```python
from build123d import *

# Parameters (mm, degrees)
BOSS_EXTRUDE1_DEPTH = 10
M10_TAPPED_HOLE1_D  = 8.5


with BuildPart() as part:
    # Sketch1 → Boss-Extrude1 (new body)
    with BuildSketch(Plane(origin=(0, 0, 0), x_dir=(1, 0, 0), z_dir=(0, 1, 0))):
        with BuildLine():
            Line((-40, -57), (40, -57))
            ThreePointArc((40, -57), (47.071067812, -54.071067812), (50, -47))
            Line((50, -47), (50, 47))
            ThreePointArc((50, 47), (47.071067812, 54.071067812), (40, 57))
            Line((40, 57), (-40, 57))
            ThreePointArc((-40, 57), (-47.071067812, 54.071067812), (-50, 47))
            Line((-50, 47), (-50, -47))
            ThreePointArc((-50, -47), (-47.071067812, -54.071067812), (-40, -57))
        make_face()
    extrude(amount=BOSS_EXTRUDE1_DEPTH)

    # M10 Tapped Hole1 (through all)
    with Locations(Plane(origin=(0, 10, 0), x_dir=(1, 0, 0), z_dir=(0, 1, 0))):
        with Locations((36, 42.5), (-36, -42.5), (-36, 42.5), (36, -42.5)):
            Hole(M10_TAPPED_HOLE1_D / 2)


solid = part.part
```
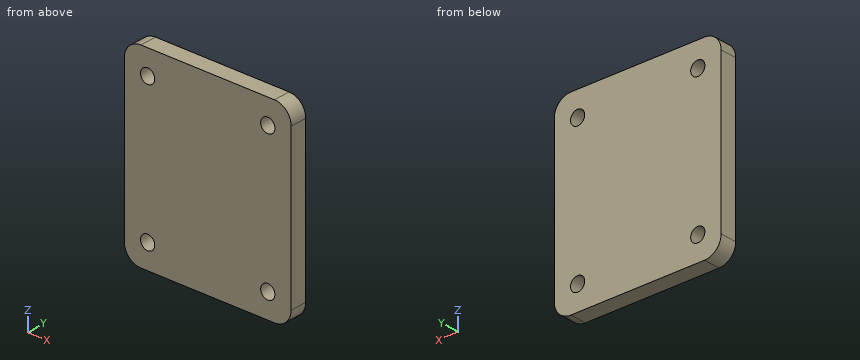
For this review, take the finished solid that the model builds, in its own axes (mm). Give positions to 0.01 mm unless a question says otherwise; leave off trailing zeros. Loops run counter-clockwise (first coordinate to the right, second up) from the corner with the lowest first, then second, coordinate; pieces in that order, holes last. Notation, with made-up numbers: M -24,0 L -12,0 A3 ccw -12,4 Z; hole C 55,11 d1. An arc over 180 degrees is marked long. One line per item, written item: value. Start each with the question number.
Q1. Clearance check with flat-ended pins moving along their axes: pin 1 Ø1 at (x, z) = (11.5, -36) entering from -Y; pin 2 Ø7.5 at (x, z) = (-36, -42.5) entering from -Y (3 decimals). State where each tip first meets the part, or that it passes through.
Q2. Add section A-A (x = 36). Give the boundary of the cut face in (y, z), and give its area (3 significant figures).
Q3. For L1, parallel to Z at x = -36, y = 2.25; L2, parallel to X at y = 3.75, z = -42.5; L3, parallel to X at y = 9.75, z = 39, list the stretches that pass through material, from the lowest coordinate up.
Q4. Add section B-B (z = 42.5). Give the boundary of the cut face in (x, y).
Q5. Add section C-C (y = 7). Give the boundary of the cut face in (x, z).
Reply:
1. pin 1: y = 0
1. pin 2: through
2. outline: M 0,-57 L 10,-57 L 10,-46.75 L 0,-46.75 Z; M 0,-38.25 L 10,-38.25 L 10,38.25 L 0,38.25 Z; M 0,46.75 L 10,46.75 L 10,57 L 0,57 Z
2. area: 970 mm²
3. L1: -57 to -46.75, -38.25 to 38.25, 46.75 to 57
3. L2: -50 to -40.25, -31.75 to 31.75, 40.25 to 50
3. L3: -50 to -38.41, -33.59 to 33.59, 38.41 to 50
4. outline: M -50,0 L -40.25,0 L -40.25,10 L -50,10 Z; M -31.75,0 L 31.75,0 L 31.75,10 L -31.75,10 Z; M 40.25,0 L 50,0 L 50,10 L 40.25,10 Z
5. outline: M -50,-47 A10 ccw -40,-57 L 40,-57 A10 ccw 50,-47 L 50,47 A10 ccw 40,57 L -40,57 A10 ccw -50,47 Z; hole C -36,-42.5 d8.5; hole C -36,42.5 d8.5; hole C 36,-42.5 d8.5; hole C 36,42.5 d8.5
